Build history of the part. All positions in model axes, mm. Round coordinates to 2 decimals unless told otherwise and drop trailing zeros. Write each loop counter-clockwise with the first axis right and the second up, starting at its lowest first coordinate (ties: lowest second). Pieces come first, ordered by that corner, then holes.
Item 1: Wall check: probe 1 along Y at (x, z) = (70, 2.3); probe 2 along X at (y, z) = (-0.75, 1.9); probe 3 along X at (y, z) = (5, 2.75). Give the ranges that are in metal, low to high.
Item 2: Band-saw the part on A-A, the plane y = 0. Write the cut outline in (x, z), then the cut area to 3 significant figures.
Item 3: Band-saw the part on B-B, the plane x = 71. Write the cut outline in (y, z), then the cut area to 3 significant figures.
Item 4: Band-saw the part on D-D, the plane x = 2. Write the cut outline in (y, z), then the cut area to 3 significant figures.
Item 5: Band-saw the part on C-C, the plane z = 0.95. Write the cut outline in (x, y), then the cut area to 3 significant figures.
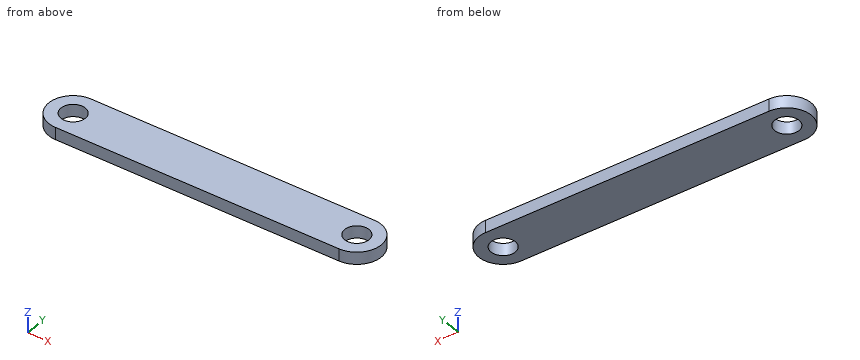
```python
from build123d import *

# Parameters (mm, degrees)
SKETCH1_R           = 3
BOSS_EXTRUDE1_DEPTH = 3


with BuildPart() as part:
    # Sketch1 → Boss-Extrude1 (new body)
    with BuildSketch(Plane.XY):
        with BuildLine():
            Line((0, 6), (70, 6))
            ThreePointArc((70, 6), (76, 0), (70, -6))
            Line((70, -6), (0, -6))
            ThreePointArc((0, -6), (-6, 0), (0, 6))
        make_face()
        Circle(SKETCH1_R, mode=Mode.SUBTRACT)
        with Locations((70, 0)):
            Circle(SKETCH1_R, mode=Mode.SUBTRACT)
    extrude(amount=BOSS_EXTRUDE1_DEPTH)


solid = part.part
```
Results:
1. probe 1: y = -6 to -3, 3 to 6
1. probe 2: x = -5.95 to -2.9, 2.9 to 67.1, 72.9 to 75.95
1. probe 3: x = -3.32 to 73.32
2. outline: (-6, 0) - (-3, 0) - (-3, 3) - (-6, 3) - close; (3, 0) - (67, 0) - (67, 3) - (3, 3) - close; (73, 0) - (76, 0) - (76, 3) - (73, 3) - close
2. area: 210 mm2
3. outline: (-5.92, 0) - (-2.83, 0) - (-2.83, 3) - (-5.92, 3) - close; (2.83, 0) - (5.92, 0) - (5.92, 3) - (2.83, 3) - close
3. area: 18.5 mm2
4. outline: (-6, 0) - (-2.24, 0) - (-2.24, 3) - (-6, 3) - close; (2.24, 0) - (6, 0) - (6, 3) - (2.24, 3) - close
4. area: 22.6 mm2
5. outline: (0, -6) - (70, -6) arc R6 ccw to (70, 6) - (0, 6) arc R6 ccw to start; hole circle Ø6 at (0, 0); hole circle Ø6 at (70, 0)
5. area: 897 mm2
